```python
from build123d import *


with BuildPart() as part:
    # 草图1 → 旋转1 (revolve)
    with BuildSketch(Plane.XY, mode=Mode.PRIVATE) as revolve_1_sk:
        Polygon((25.3, 25.5), (25.3, 20.5), (0.8, 20.5), (0.8, 13.5), (0, 13.5), (0, 10), (27.5, 10), (27.5, 13.5), (4.3, 13.5), (4.3, 18.5), (27.5, 18.5), (27.5, 25.5), align=None)
    revolve(revolve_1_sk.sketch.rotate(Axis((0, 0, 0), (1, 0, 0)), 90), axis=Axis((0, 0, 0), (1, 0, 0)))


solid = part.part
```
Can you work these out from the model? Positions are in its coordinate system, mm. A direction names the side the tool comes from. Round coordinates to 2 decimals unless told otherwise and drop trailing zeros. Loops run counter-clockwise (first coordinate to the right, second up) from the corner with the lowest first, then second, coordinate; pieces in that order, holes last. Notation, with made-up numbers: M 35,51.5 L 43,51.5 A26 cw 43,69.5 Z; hole C 83.5,-3 d2. An arc over 180 degrees is marked long. Answer as a JSON object with one key per item and string values. Group by question number.
Q1. Will these pins go through, and if not, where does the flat tip stop? pin 1 (3 mm diameter, centred on x = 14, y = 7.5, fed in from -Z); pin 2 (3 mm diameter, centred on x = 24, y = -3, fed in from +Z); pin 3 (4 mm diameter, centred on x = 7.5, z = 3, fed in from +Y).
Q2. Imagine slicing it at A-A, the plane z = 0. Please give me the cut outline in (x, y), then the cut area to 3 significant figures.
Q3. Imagine slicing it at C-C, the plane x = 17.5. Please give me the cut outline in (y, z), then the cut area to 3 significant figures.
Q4. On a 3-axis mill with a long thin cutter (end or side, diameter ignored), from which of +Z, -Z, +X, -X, +Y, -Y can I reach the whole of each face in a straight line? I mean faces 5 (the flat face through (4.3, 14, -1)), 6 (the flat face through (27.5, 5, 9)), 7 (the cylindrical face through (12.878, 7.852, 18.937)). Say none if no direction works.
Q5. Imagine slicing it at D-D, the plane y = 11. Please give me the cut outline in (x, z), then the cut area to 3 significant figures.
Q6. We'd pull the mould along Y, two halves only. Please class faces 1 (the cylindrical face through (0.39, 13.18, -2.93)), 2 (the cylindrical face through (14, 0, -10)), 3 (the flat face through (25.3, -21, 2)), 4 (the cylindrical face through (16.06, 16.41, 8.54)): +Y half, -Y half, draft (parallel to the pull), parting line (faces both ways), or undercut.
Q7. Please list where these lines run through material, in increasing order: L1, parallel to Y at x = 18.75, z = 0; L2, parallel to Y at x = 9, z = -7.5; L3, parallel to Z at x = 17, y = -0.5.
Findings:
{
 "1": {"pin 1": "stops at z = -19.6", "pin 2": "stops at z = 25.4", "pin 3": "stops at y = 20.48"},
 "2": {"outline": "M 0,-13.5 L 0.8,-13.5 L 0.8,-20.5 L 25.3,-20.5 L 25.3,-25.5 L 27.5,-25.5 L 27.5,-18.5 L 4.3,-18.5 L 4.3,-13.5 L 27.5,-13.5 L 27.5,-10 L 0,-10 Z; M 0,10 L 27.5,10 L 27.5,13.5 L 4.3,13.5 L 4.3,18.5 L 27.5,18.5 L 27.5,25.5 L 25.3,25.5 L 25.3,20.5 L 0.8,20.5 L 0.8,13.5 L 0,13.5 Z", "area": "356 mm2"},
 "3": {"outline": "C 0,0 d41; C 0,0 d27; hole C 0,0 d37; hole C 0,0 d20", "area": "503 mm2"},
 "4": {"face 5": "+X", "face 6": "+Z, -Z, +X, +Y, -Y", "face 7": "-X"},
 "5": {"outline": "M 0,-7.83 L 0.8,-7.83 L 0.8,-17.3 L 25.3,-17.3 L 25.3,-23.01 L 27.5,-23.01 L 27.5,-14.87 L 4.3,-14.87 L 4.3,-7.83 L 27.5,-7.83 L 27.5,7.83 L 4.3,7.83 L 4.3,14.87 L 27.5,14.87 L 27.5,23.01 L 25.3,23.01 L 25.3,17.3 L 0.8,17.3 L 0.8,7.83 L 0,7.83 Z", "area": "634 mm2"},
 "6": {"face 1": "parting line", "face 2": "undercut", "face 3": "draft", "face 4": "undercut"},
 "7": {"L1": "y = -20.5 to -18.5, -13.5 to -10, 10 to 13.5, 18.5 to 20.5", "L2": "y = -19.08 to -16.91, -11.22 to -6.61, 6.61 to 11.22, 16.91 to 19.08", "L3": "z = -20.49 to -18.49, -13.49 to -9.99, 9.99 to 13.49, 18.49 to 20.49"}
}
